```python
from build123d import *

# Parameters (mm, degrees)
SKETCH_1_W                  = 110
SKETCH_1_H                  = 105
EXTRUDE_1_DEPTH             = 5
CUT_EXTRUDE_1_DEPTH         = 10
CHAMFER_1_SIZE              = 5
HOLE_WIZARD_M5_1_AT_2_COUNT = 2
HOLE_WIZARD_M5_1_AT_2_PITCH = 80


with BuildPart() as part:
    # 草图1 → 凸台-拉伸1 (new, symmetric)
    with BuildSketch(Plane(origin=(0, 0, 0), x_dir=(1, 0, 0), z_dir=(0, 1, 0))):
        Rectangle(SKETCH_1_W, SKETCH_1_H)
    extrude(amount=EXTRUDE_1_DEPTH, both=True)

    # 草图2 → 切除-拉伸1 (cut)
    with BuildSketch(Plane(origin=(0, 5, 0), x_dir=(1, 0, 0), z_dir=(0, 1, 0))):
        with BuildLine():
            Line((55, 52.5), (-30, 52.5))
            Line((-30, 52.5), (-30, -7.5))
            ThreePointArc((-30, -7.5), (-24.142135624, -21.642135624), (-10, -27.5))
            Line((-10, -27.5), (55, -27.5))
            Line((55, -27.5), (55, 52.5))
        make_face()
    extrude(amount=-CUT_EXTRUDE_1_DEPTH, mode=Mode.SUBTRACT)

    # 倒角1
    chamfer_1_edges = [part.edges().sort_by_distance(p)[0] for p in [
        (-30, 0, -52.5),
        (55, 0, 27.5),
    ]]
    chamfer(chamfer_1_edges, length=CHAMFER_1_SIZE)

    # 草图4 → M5 螺纹孔1 (revolve, cut)
    with BuildSketch(Plane(origin=(-55, 0, 37.5), x_dir=(0, 0, 1), z_dir=(0, 1, 0))):
        Polygon((0, 0), (0, 13.6618073), (2.1, 12.4), (2.1, 0), align=None)
    hole_wizard_m5_1 = revolve(axis=Axis((-61.35, 0, 37.5), (1, 0, 0)), mode=Mode.SUBTRACT)

    # M5 螺纹孔1 at 2: M5 螺纹孔1 ×2
    with Locations(*[(0, 0, -i * HOLE_WIZARD_M5_1_AT_2_PITCH) for i in range(1, HOLE_WIZARD_M5_1_AT_2_COUNT)]):
        add(hole_wizard_m5_1, mode=Mode.SUBTRACT)

    # 镜向1: M5 螺纹孔1 across plane
    add(hole_wizard_m5_1.mirror(Plane(origin=(-1.25, 0, -1.25), x_dir=(-0.7071067811865478, 0, 0.7071067811865472), z_dir=(-0.7071067811865475, 0, -0.7071067811865477))), mode=Mode.SUBTRACT)

    # 镜向1 copy 1 sketch → 镜向1 copy 1 (revolve, cut)
    with BuildSketch(Plane(origin=(40, 0, 52.5), x_dir=(-1, 0, 0), z_dir=(0, 1, 0))):
        Polygon((0, 0), (0, -13.6618073), (2.1, -12.4), (2.1, 0), align=None)
    revolve(axis=Axis((40, 0, 58.85), (0, 0, 1)), mode=Mode.SUBTRACT)


solid = part.part
```
Design review of the part built by this model. Coordinates are the model's own, in mm. A direction names the side the tool comes from. Give positions to 0.01 mm unless a question says otherwise; leave off trailing zeros. Order: outer loops, then holes, each group sorted by start corner. A loop starts at its lowest first (then second) coordinate and runs counter-clockwise, first axis right, second up. Notation, with made-up numbers: (-16, 68) - (1, 68) arc R23 cw to (1, 81) - close; hole circle Ø10 at (14, -23.75). An arc over 180 degrees is marked (long way). Use a Markdown table: item, result. Add a question column.
(1) Machinability: for faces 1 (the face through (-55, 0, 1)), 2 (the face through (-48.89, -0.09, 35.4)), 3 (the face through (-25, 5, 23)), 4 (the face through (42.1, -0.09, 46.39)), 5 (the face through (-30, 0, -20)), which of the approach directions +Z, -Z, +X, -X, +Y, -Y give a long, thin tool a straight path to every point of the face, cutting with its end or side? Answer none if there is none.
(2) Add section A-A on x = -45.5. Give the boundary of the cut face in (y, z).
(3) Wall thickness on probe 1 along X at (y, z) = (0, 43); probe 2 along Y at (x, z) = (40, 44); probe 3 along Z at (x, y) = (-4, -0.75): over which ranges is each line inside the solid? List them lowest first. Write a range as [from, to].
(4) Add section C-C on x = 46. Give the boundary of the cut face in (y, z).
(5) Mouldability with a two-part tool opening along Z and no side actions: class faces 6 (the face through (20, 0, 27.5)), 7 (the face through (39.65, -0.11, 39.06)), 8 (the face through (-41.557, -0.016, 37.136)) as +Z half, -Z half, draft (parallel to the pull), parting line (faces both ways), or undercut.
(6) Add section B-B on z = -46. Give the boundary of the cut face in (x, y).
(7) Clearance check with flat-ended pins moving along their axes: P1, Ø1.5, axis at x = 29, y = 1.5, coming from the -Z side; P2, Ø5, axis at y = 0, z = 37.5, coming from the -X side; P3, Ø5, axis at y = -1, z = -28.5, coming from the +X side; P4, Ø4, axis at x = -40, y = 0, coming from the +Z side. State where each tip first meets the part, or that it passes through.
Report:
| question | item | result |
|---|---|---|
| 1 | face 1 | +Z, -Z, -X, +Y, -Y |
| 1 | face 2 | -X |
| 1 | face 3 | +Z, -Z, +X, -X, +Y |
| 1 | face 4 | +Z |
| 1 | face 5 | -Z, +X, +Y, -Y |
| 2 | outline | (-5, -52.5) - (5, -52.5) - (5, 52.5) - (-5, 52.5) - close; hole circle Ø4.2 at (0, -42.5); hole circle Ø4.2 at (0, 37.5) |
| 3 | probe 1 | x = [-55, -42.1], [-37.9, 37.9], [42.1, 55] |
| 3 | probe 2 | y = [-5, -2.1], [2.1, 5] |
| 3 | probe 3 | z = [27.5, 52.5] |
| 4 | outline | (-5, 27.5) - (5, 27.5) - (5, 52.5) - (-5, 52.5) - close |
| 5 | face 6 | -Z half |
| 5 | face 7 | +Z half |
| 5 | face 8 | undercut |
| 6 | outline | (-55, -5) - (-30, -5) - (-30, 5) - (-55, 5) - close |
| 7 | P1 | stops at z = 27.5 |
| 7 | P2 | stops at x = -55 |
| 7 | P3 | stops at x = -30 |
| 7 | P4 | stops at z = 40.04 |
